The listing builds one solid part. Answer for the finished solid, in the listing's coordinates (mm). Face numbers are marked on the shaded views. A direction names the side the tool comes from. Give positions to 0.01 mm unless a question says otherwise; leave off trailing zeros. Order: outer loops, then holes, each group sorted by start corner. A loop starts at its lowest first (then second) coordinate and runs counter-clockwise, first axis right, second up. Notation, with made-up numbers: (71.5, 20.5) - (99.5, 20.5) arc R31 cw to (99.5, 47.5) - close; hole circle Ø11 at (-26, 60). An arc over 180 degrees is marked (long way). Write each question's results on one line, items separated by ' | '. Start each with the question number.
1. Section D-D (x = 2.5) is taken. Give the vertices of the cut face in (y, z).
2. Flat-ended cylindrical pins translate along their axes: pin 1 (8 mm diameter, centred on x = -3.5, y = 6, fed in from -Z); pin 2 (1.2 mm diameter, centred on x = 18.5, z = -2.5, fed in from +Y); pin 3 (1.7 mm diameter, centred on x = 18, z = -1, fed in from -Y). Find the tip coordinate at first contact, or state that the pin passes through.
3. Which of the six approach directions +Z, -Z, +X, -X, +Y, -Y give full straight-line access (tool end or side, diameter ignored) to the marked faces 1 and 2?
4. Section A-A (y = 0) is taken. Give the vertices of the cut face in (x, z).
5. Section C-C (x = 16.5) is taken. Give the vertices of the cut face in (y, z).
6. Find the intervals of material crossed by L1, parallel to X at y = 0.5, z = 10; L2, parallel to X at y = -5, z = 5.5; L3, parallel to Z at x = 13, y = 7.25, in increasing order.
7. Section B-B (z = 0) is taken. Give the vertices of the cut face in (x, y).
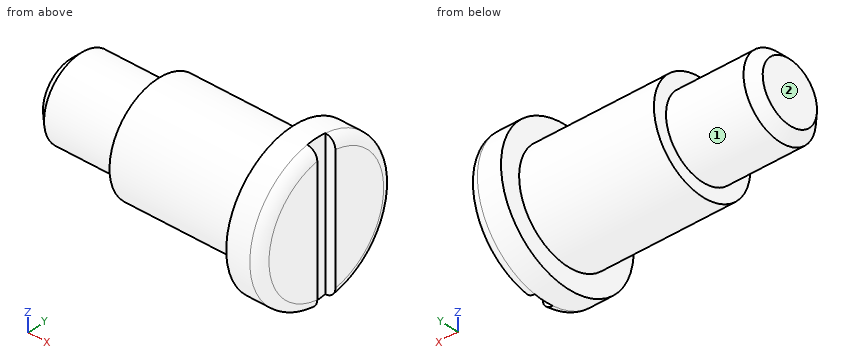
from build123d import *

# Parameters (mm, degrees)
SKETCH2_W          = 26.278844289
SKETCH2_H          = 3
CUT_EXTRUDE1_DEPTH = 1.5
FILLET1_R          = 1.5
CHAMFER1_SIZE      = 1.5


with BuildPart() as part:
    # Sketch1 → Revolve1 (revolve)
    with BuildSketch(Plane(origin=(0, 0, 0), x_dir=(1, 0, 0), z_dir=(0, 1, 0)), mode=Mode.PRIVATE) as revolve1_sk:
        Polygon((-19, 0), (-19, 6), (-6, 6), (-6, 8), (14, 8), (14, 11), (19, 11), (19, 0), align=None)
    revolve(revolve1_sk.sketch.rotate(Axis((-19, 0, 0), (1, 0, 0)), 180), axis=Axis((-19, 0, 0), (1, 0, 0)))

    # Sketch2 → Cut-Extrude1 (cut)
    with BuildSketch(Plane(origin=(19, 0, 0), x_dir=(0, 0, -1), z_dir=(1, 0, 0))):
        with Locations((0.853209231, 0)):
            Rectangle(SKETCH2_W, SKETCH2_H)
    extrude(amount=-CUT_EXTRUDE1_DEPTH, mode=Mode.SUBTRACT)

    # Fillet1
    fillet1_edges = [part.edges().sort_by_distance(p)[0] for p in [
        (19, -11, 0),
        (19, 11, 0),
    ]]
    fillet(fillet1_edges, radius=FILLET1_R)

    # Chamfer1
    chamfer1_edges = [part.edges().sort_by_distance(p)[0] for p in [
        (-19, 0, -6),
    ]]
    chamfer(chamfer1_edges, length=CHAMFER1_SIZE)


solid = part.part
Reported:
1) outline: circle Ø16 at (0, 0)
2) pin 1: z = -7.75 | pin 2: y = 10.7 | pin 3: y = -11
3) face 1: -X | face 2: +Z, -Z, -X, +Y, -Y
4) outline: (-19, -4.5) - (-17.5, -6) - (-6, -6) - (-6, -8) - (14, -8) - (14, -11) - (17.5, -11) - (17.5, 11) - (14, 11) - (14, 8) - (-6, 8) - (-6, 6) - (-17.5, 6) - (-19, 4.5) - close
5) outline: circle Ø22 at (0, 0)
6) L1: 14 to 17.5 | L2: -6 to 19 | L3: -3.38 to 3.38
7) outline: (-19, -4.5) - (-17.5, -6) - (-6, -6) - (-6, -8) - (14, -8) - (14, -11) - (17.5, -11) arc R1.5 ccw to (19, -9.5) - (19, -1.5) - (17.5, -1.5) - (17.5, 1.5) - (19, 1.5) - (19, 9.5) arc R1.5 ccw to (17.5, 11) - (14, 11) - (14, 8) - (-6, 8) - (-6, 6) - (-17.5, 6) - (-19, 4.5) - close
